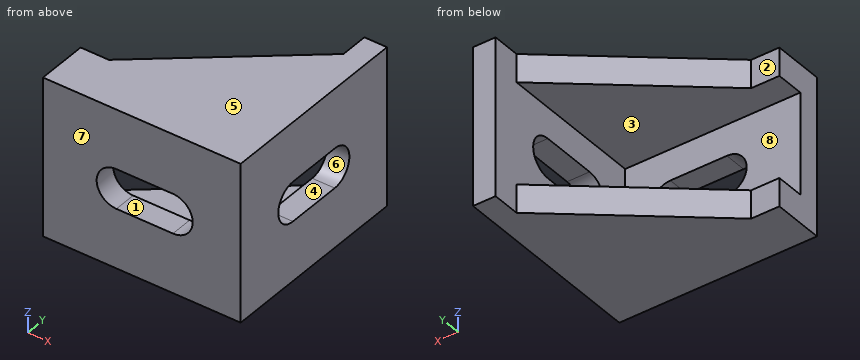
from build123d import *

# Parameters (mm, degrees)
SKETCH_1_W          = 4
SKETCH_1_H          = 31
SKETCH_1_H_2        = 4
SKETCH_1_W_2        = 31
EXTRUDE_1_DEPTH     = 14
EXTRUDE_2_DEPTH     = 5
CUT_EXTRUDE_1_DEPTH = 5
CUT_EXTRUDE_2_DEPTH = 5


with BuildPart() as part:
    # 草图1 → 凸台-拉伸1 (new, symmetric)
    with BuildSketch(Plane.XY):
        with Locations((0, 2)):
            Rectangle(SKETCH_1_W, SKETCH_1_H)
        with Locations((0, -15.5)):
            Rectangle(SKETCH_1_W, SKETCH_1_H_2)
        with Locations((-17.5, -15.5)):
            Rectangle(SKETCH_1_W_2, SKETCH_1_H_2)
    extrude(amount=EXTRUDE_1_DEPTH, both=True)

    # 草图2 → 凸台-拉伸2 (add)
    with BuildSketch(Plane(origin=(0, 0, -14), x_dir=(-1, 0, 0), z_dir=(0, 0, -1))):
        Polygon((2, 12.5), (28, -8.5), (33, -8.5), (33, -13.5), (2, -13.5), align=None)
    extrude_2 = extrude(amount=-EXTRUDE_2_DEPTH)

    # 镜向1: 凸台-拉伸2 across plane
    add(extrude_2.mirror(Plane.XY))

    # 草图3 → 切除-拉伸1 (cut)
    with BuildSketch(Plane.ZY.offset(2)):
        with BuildLine():
            Line((-3.5, -5), (-3.5, 5))
            ThreePointArc((-3.5, 5), (0, 8.5), (3.5, 5))
            Line((3.5, 5), (3.5, -5))
            ThreePointArc((3.5, -5), (0, -8.5), (-3.5, -5))
        make_face()
    extrude(amount=-CUT_EXTRUDE_1_DEPTH, mode=Mode.SUBTRACT)

    # 草图4 → 切除-拉伸2 (cut)
    with BuildSketch(Plane(origin=(0, -13.5, 0), x_dir=(1, 0, 0), z_dir=(0, 1, 0))):
        with BuildLine():
            Line((-20, 3.5), (-10, 3.5))
            ThreePointArc((-10, 3.5), (-6.5, 0), (-10, -3.5))
            Line((-10, -3.5), (-20, -3.5))
            ThreePointArc((-20, -3.5), (-23.5, 0), (-20, 3.5))
        make_face()
    extrude(amount=-CUT_EXTRUDE_2_DEPTH, mode=Mode.SUBTRACT)


solid = part.part
Part model, mm, in its own coordinate system. Face numbers are marked on the shaded views. A direction names the side the tool comes from. Give positions to 0.01 mm unless a question says otherwise; leave off trailing zeros. Order: outer loops, then holes, each group sorted by start corner. A loop starts at its lowest first (then second) coordinate and runs counter-clockwise, first axis right, second up. Notation, with made-up numbers: (14, 79) -> (66, 79) arc R28 ccw to (66, 103) -> close; hole circle Ø1 at (82, -27). An arc over 180 degrees is marked (long way). Use one line per item in the form item = value.
(1) Drill centre lines: line 1 (Z direction, x = -25, y = -6.5); line 2 (Z direction, x = -18, y = -14.5); line 3 (Y direction, x = -16.5, z = -6). Where is each one in solid material? Low to high. Write a range as from..to.
Solution:
line_1 = -14..-9, 9..14
line_2 = -14..-3.5, 3.5..14
line_3 = -17.5..-13.5
(2) Saw through at A-A (z = 0). Write the cut outline in (x, y).
Solution:
outline = (-33, -17.5) -> (-23.5, -17.5) -> (-23.5, -13.5) -> (-33, -13.5) -> close; (-6.5, -17.5) -> (2, -17.5) -> (2, -8.5) -> (-2, -8.5) -> (-2, -13.5) -> (-6.5, -13.5) -> close; (-2, 8.5) -> (2, 8.5) -> (2, 17.5) -> (-2, 17.5) -> close
(3) Tool access for the marked faces 1, 2, 3 and 4: list every direction of +Z, -Z, +X, -X, +Y, -Y with a clear straight run to the whole face (end or side of a thin tool).
Solution:
face_1 = +Y, -Y
face_2 = +Z, -Z, -X, +Y
face_3 = -X, +Y
face_4 = +X, -X
(4) Pull direction Y, two halves, no side cores. Call the marked faces 5, 6, 7 and 8: +Y half, -Y half, draft (parallel to the pull), parting line (faces both ways), or undercut.
Solution:
face_5 = draft
face_6 = undercut
face_7 = -Y half
face_8 = +Y half
(5) Saw through at C-C (y = 6). Write the cut outline in (x, z).
Solution:
outline = (-10.05, -14) -> (2, -14) -> (2, -3.35) -> (-2, -3.35) -> (-2, -9) -> (-10.05, -9) -> close; (-10.05, 9) -> (-2, 9) -> (-2, 3.35) -> (2, 3.35) -> (2, 14) -> (-10.05, 14) -> close
(6) Flat gauge pins, fed straight in: P1, Ø5.5, axis at x = -31.5, z = -12, coming from the +Y side; P2, Ø9, axis at x = -10.5, z = 1.5, coming from the +Y side; P3, Ø5, axis at y = 8, z = 8.5, coming from the -X side. Where does each tip first touch, or does it go through?
Solution:
P1 = -8.5
P2 = -13.5
P3 = -10.6
(7) Saw through at B-B (x = -19). Write the cut outline in (y, z).
Solution:
outline = (-17.5, -14) -> (-1.23, -14) -> (-1.23, -9) -> (-13.5, -9) -> (-13.5, -3.5) -> (-17.5, -3.5) -> close; (-17.5, 3.5) -> (-13.5, 3.5) -> (-13.5, 9) -> (-1.23, 9) -> (-1.23, 14) -> (-17.5, 14) -> close
(8) Saw through at D-D (z = -11). Write the cut outline in (x, y).
Solution:
outline = (-33, -17.5) -> (2, -17.5) -> (2, 17.5) -> (-2, 17.5) -> (-2, 12.5) -> (-28, -8.5) -> (-33, -8.5) -> close
